Check sheet for the modelled part. Datum: model origin and axes. Units: mm. Face numbers are marked on the shaded views. A direction names the side the tool comes from. Round coordinates to 2 decimals unless told otherwise and drop trailing zeros. Loops run counter-clockwise (first coordinate to the right, second up) from the corner with the lowest first, then second, coordinate; pieces in that order, holes last. Notation, with made-up numbers: (4, -3.75) -> (19, -3.75) arc R37 ccw to (19, 32.25) -> close; hole circle Ø4 at (56.5, 34.5). An arc over 180 degrees is marked (long way). Return JSON: item names as keys, results as strings.
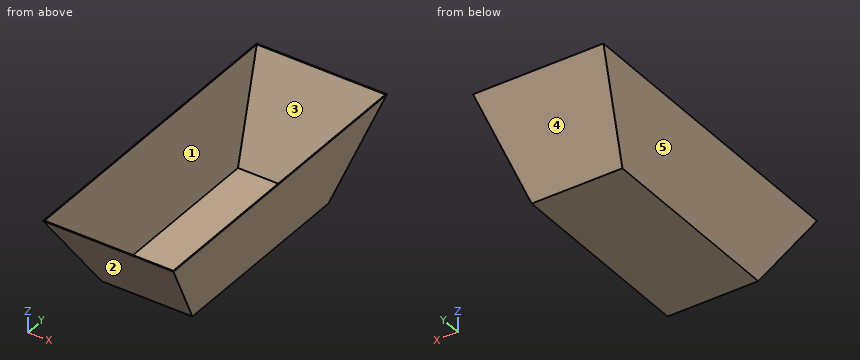
from build123d import *

# Parameters (mm, degrees)
SKETCH1_W           = 460
SKETCH1_H           = 1100
BOSS_EXTRUDE1_DEPTH = 300
CUT_EXTRUDE1_DEPTH  = 778.238702073
CUT_EXTRUDE3_DEPTH  = 949
SHELL1_T            = -3


with BuildPart() as part:
    # Sketch1 → Boss-Extrude1 (new body)
    with BuildSketch(Plane.XY):
        Rectangle(SKETCH1_W, SKETCH1_H)
    extrude(amount=-BOSS_EXTRUDE1_DEPTH)

    # Sketch3 → Cut-Extrude1 (cut, through all)
    with BuildSketch(Plane(origin=(230, 0, 0), x_dir=(0, 0, -1), z_dir=(1, 0, 0))):
        Polygon((0, 550), (300, 350), (300, 550), align=None)
        Polygon((300, -550), (0, -550), (300, -350), align=None)
    extrude(amount=-CUT_EXTRUDE1_DEPTH, mode=Mode.SUBTRACT)

    # Sketch6 → Cut-Extrude3 (cut, symmetric)
    with BuildSketch(Plane(origin=(0, 0, 0), x_dir=(1, 0, 0), z_dir=(0, 1, 0))):
        Polygon((-230, 0), (-160, 300), (-230, 300), align=None)
        Polygon((230, 300), (230, 0), (160, 300), align=None)
    extrude(amount=CUT_EXTRUDE3_DEPTH, both=True, mode=Mode.SUBTRACT)

    # Shell1
    shell1_openings = [part.faces().sort_by_distance(p)[0] for p in [
        (0, 0, 0),
    ]]
    offset(amount=SHELL1_T, openings=shell1_openings, kind=Kind.INTERSECTION)


solid = part.part
Q1. Section check A-A (x = 92). Record the boundary of the cut face in (y, z).
Results list:
{"outline": "(-550, 0) -> (-350, -300) -> (350, -300) -> (550, 0) -> (546.39, 0) -> (348.39, -297) -> (-348.39, -297) -> (-546.39, 0) -> close"}
Q2. Section check D-D (z = -255). Record the boundary of the cut face in (x, y).
Results list:
{"outline": "(-170.5, -380) -> (170.5, -380) -> (170.5, 380) -> (-170.5, 380) -> close; hole (-167.42, -376.39) -> (167.42, -376.39) -> (167.42, 376.39) -> (-167.42, 376.39) -> close"}
Q3. Tool access check on the marked faces 1 and 2. Record the directions out of +Z, -Z, +X, -X, +Y, -Y that give a thin tool (end or side, any length) a straight path to the whole face; none if there is none.
Results list:
{"face 1": "+Z", "face 2": "-Z, +X, -X, -Y"}
Q4. Draft check along Y on the marked faces 3, 4 and 5. Enter one of: released by +Y, released by -Y, zero draft, split by the parting line, or undercut.
Results list:
{"face 3": "undercut", "face 4": "released by +Y", "face 5": "zero draft"}
Q5. Section check B-B (z = -151.5). Record the boundary of the cut face in (x, y), then the cut area to 3 significant figures.
Results list:
{"outline": "(-194.65, -449) -> (194.65, -449) -> (194.65, 449) -> (-194.65, 449) -> close; hole (-191.57, -445.39) -> (191.57, -445.39) -> (191.57, 445.39) -> (-191.57, 445.39) -> close", "area": "8,300 mm^2"}
Q6. Go/stop test with flat-tipped pins: pin 1 (3 mm diameter, centred on y = 14.5, z = -71, fed in from -X); pin 2 (1 mm diameter, centred on y = -221, z = -113, fed in from -X); pin 3 (5 mm diameter, centred on x = -124.5, y = -407.5, fed in from -Z). Record where each tip stops, or that it passes through.
Results list:
{"pin 1": "x = -213.78", "pin 2": "x = -203.75", "pin 3": "z = -217.5"}
Q7. Material ranges on line 1 (Z direction, x = -22.5, y = 212); line 2 (Y direction, x = -20, z = -139); line 3 (Y direction, x = 90.5, z = -154), recorded low to high.
Results list:
{"line 1": "-300 to -297", "line 2": "-457.33 to -453.73, 453.73 to 457.33", "line 3": "-447.33 to -443.73, 443.73 to 447.33"}
Q8. Section check C-C (y = -144). Record the boundary of the cut face in (x, z).
Results list:
{"outline": "(-230, 0) -> (-160, -300) -> (160, -300) -> (230, 0) -> (226.92, 0) -> (157.62, -297) -> (-157.62, -297) -> (-226.92, 0) -> close"}
